```python
from build123d import *

# Parameters (mm, degrees)
SKETCH1_R           = 35
BOSS_EXTRUDE1_DEPTH = 10
SKETCH2_R           = 25
BOSS_EXTRUDE2_DEPTH = 50
CHAMFER1_SIZE       = 3
SKETCH3_R           = 9
CUT_EXTRUDE1_DEPTH  = 11
SKETCH4_R           = 5.5
CUT_EXTRUDE2_DEPTH  = 76


with BuildPart() as part:
    # Sketch1 → Boss-Extrude1 (new body)
    with BuildSketch(Plane(origin=(0, 0, 0), x_dir=(1, 0, 0), z_dir=(0, 1, 0))):
        with Locations(Location((0, 0, 0), (0, 0, 270))):
            Circle(SKETCH1_R)
    extrude(amount=BOSS_EXTRUDE1_DEPTH)

    # Sketch2 → Boss-Extrude2 (add)
    with BuildSketch(Plane(origin=(0, 10, 0), x_dir=(1, 0, 0), z_dir=(0, 1, 0))):
        with Locations(Location((0, 0, 0), (0, 0, 270))):
            Circle(SKETCH2_R)
    extrude(amount=BOSS_EXTRUDE2_DEPTH)

    # Chamfer1
    chamfer1_edges = [part.edges().sort_by_distance(p)[0] for p in [
        (0, 60, -25),
    ]]
    chamfer(chamfer1_edges, length=CHAMFER1_SIZE)

    # Sketch3 → Cut-Extrude1 (cut)
    with BuildSketch(Plane(origin=(0, 60, 0), x_dir=(1, 0, 0), z_dir=(0, 1, 0))):
        with Locations(Location((0, 0, 0), (0, 0, 270))):
            Circle(SKETCH3_R)
    extrude(amount=-CUT_EXTRUDE1_DEPTH, mode=Mode.SUBTRACT)

    # Sketch4 → Cut-Extrude2 (cut)
    with BuildSketch(Plane(origin=(0, 49, 0), x_dir=(1, 0, 0), z_dir=(0, 1, 0))):
        with Locations(Location((0, 0, 0), (0, 0, 270))):
            Circle(SKETCH4_R)
    extrude(amount=-CUT_EXTRUDE2_DEPTH, mode=Mode.SUBTRACT)


solid = part.part
```
The model under review builds one solid part; all positions refer to its coordinate system, in mm. A direction names the side the tool comes from. Round coordinates to 2 decimals unless told otherwise and drop trailing zeros. Write each loop counter-clockwise with the first axis right and the second up, starting at its lowest first coordinate (ties: lowest second). Pieces come first, ordered by that corner, then holes. Notation, with made-up numbers: (-18.75, 51.5) - (19.25, 51.5) arc R8 cw to (19.25, 63.5) - close; hole circle Ø11 at (77.25, -16.75). An arc over 180 degrees is marked (long way). Use one line per item in the form item = value.
Q1. Consider section C-C (y = 52). State the section outline as (x, z) points, and give its area (3 significant figures).
Answer key:
outline = circle Ø50 at (0, 0); hole circle Ø18 at (0, 0)
area = 1,710 mm2
Q2. For line 1 (X direction, y = 56.5, z = 0); line 2 (X direction, y = 24.5, z = 0); line 3 (Y direction, x = 11.5, z = 32), list the stretches that pass through material, from the lowest coordinate up. Write a range as [from, to].
Answer key:
line_1 = [-25, -9], [9, 25]
line_2 = [-25, -5.5], [5.5, 25]
line_3 = [0, 10]
Q3. Draft analysis for pull direction Z (two halves, no side actions). For faces 1 (the flat face through (8, 10, -24)), 2 (the conical face through (-21.619, 59.854, -4.801)), 3 (the cylindrical face through (-5.37, 24.84, -1.19)), state which applies: +Z half, -Z half, draft (parallel to the pull), parting line (faces both ways), or undercut.
Answer key:
face_1 = draft
face_2 = parting line
face_3 = undercut
Q4. Consider section B-B (x = 0). State the section outline as (y, z) points, and give its area (3 significant figures).
Answer key:
outline = (0, -35) - (10, -35) - (10, -25) - (57, -25) - (60, -22) - (60, -9) - (49, -9) - (49, -5.5) - (0, -5.5) - close; (0, 5.5) - (49, 5.5) - (49, 9) - (60, 9) - (60, 22) - (57, 25) - (10, 25) - (10, 35) - (0, 35) - close
area = 2,450 mm2
Q5. Consider section D-D (z = -30). State the section outline as (x, y) points.
Answer key:
outline = (-18.03, 0) - (18.03, 0) - (18.03, 10) - (-18.03, 10) - close
Q6. Insertion check: pin 1 Ø2 at (x, y) = (11.5, 48.5) entering from -Z; pin 2 Ø2 at (x, z) = (-13, -27.5) entering from +Y; pin 3 Ø14.5 at (x, z) = (0, 0) entering from +Y; pin 4 Ø20 at (x, z) = (4, 2.5) entering from +Y. Each pin has a flat end and moves straight along its axis. Give the tip position at first contact, or say it passes through.
Answer key:
pin_1 = -22.69
pin_2 = 10
pin_3 = 49
pin_4 = 60
Q7. Consider section A-A (z = 0). State the section outline as (x, y) points, and give its area (3 significant figures).
Answer key:
outline = (-35, 0) - (-5.5, 0) - (-5.5, 49) - (-9, 49) - (-9, 60) - (-22, 60) - (-25, 57) - (-25, 10) - (-35, 10) - close; (5.5, 0) - (35, 0) - (35, 10) - (25, 10) - (25, 57) - (22, 60) - (9, 60) - (9, 49) - (5.5, 49) - close
area = 2,450 mm2
Q8. Tool access review of faces 4 (the flat face through (-4, 49, -4)), 5 (the flat face through (-7, 0, 0)): name each direction out of +Z, -Z, +X, -X, +Y, -Y from which nothing blocks a thin tool from reaching the whole face with its end or side.
Answer key:
face_4 = +Y
face_5 = +Z, -Z, +X, -X, -Y
